```python
from build123d import *

# Parameters (mm, degrees)
BOSS_EXTRUDE1_DEPTH       = 28
CHAMFER1_SIZE             = 2
M8X1_0_TAPPED_HOLE1_D     = 7
M8X1_0_TAPPED_HOLE1_DEPTH = 13
M8X1_0_TAPPED_HOLE1_TIP   = 2.103012167
HOLE2_D                   = 9
SKETCH15_R                = 32.5
CUT_EXTRUDE3_DEPTH        = 2.5
CUT_EXTRUDE4_START        = -2.5
SKETCH16_R                = 32.5
CUT_EXTRUDE4_DEPTH        = 2.5
HOLE3_D                   = 4


with BuildPart() as part:
    # Sketch1 → Boss-Extrude1 (new body)
    with BuildSketch(Plane.XY):
        with BuildLine():
            Line((-50, 24), (-33, 24))
            Line((-33, 24), (-33, 47))
            Line((-33, 47), (33, 47))
            Line((33, 47), (33, 24))
            Line((33, 24), (50, 24))
            Line((50, 24), (50, 0))
            Line((50, 0), (30, 0))
            ThreePointArc((30, 0), (0, 30), (-30, 0))
            Line((-30, 0), (-50, 0))
            Line((-50, 0), (-50, 24))
        make_face()
    extrude(amount=BOSS_EXTRUDE1_DEPTH)

    # Chamfer1
    chamfer1_edges = [part.edges().sort_by_distance(p)[0] for p in [
        (-50, 24, 14),
        (-33, 47, 14),
        (33, 47, 14),
        (50, 24, 14),
    ]]
    chamfer(chamfer1_edges, length=CHAMFER1_SIZE)

    # M8x1.0 Tapped Hole1
    with Locations(Plane(origin=(0, 47, 0), x_dir=(1, 0, 0), z_dir=(0, 1, 0))):
        with Locations((0, -14)):
            Hole(M8X1_0_TAPPED_HOLE1_D / 2, depth=M8X1_0_TAPPED_HOLE1_DEPTH)
            with Locations((0, 0, -(M8X1_0_TAPPED_HOLE1_DEPTH + M8X1_0_TAPPED_HOLE1_TIP / 2))):  # 118° drill point
                Cone(0, M8X1_0_TAPPED_HOLE1_D / 2, M8X1_0_TAPPED_HOLE1_TIP, mode=Mode.SUBTRACT)

    # Hole2 (through all)
    with Locations(Plane(origin=(0, 24, 0), x_dir=(1, 0, 0), z_dir=(0, 1, 0))):
        with Locations((-41, -14), (41, -14)):
            Hole(HOLE2_D / 2)

    # Sketch15 → Cut-Extrude3 (cut)
    with BuildSketch(Plane(origin=(0, 0, 0), x_dir=(-1, 0, 0), z_dir=(0, 0, -1))):
        Circle(SKETCH15_R)
    extrude(amount=-CUT_EXTRUDE3_DEPTH, mode=Mode.SUBTRACT)

    # Sketch16 → Cut-Extrude4 (cut)
    with BuildSketch(Plane.XY.offset(28).offset(CUT_EXTRUDE4_START)):
        Circle(SKETCH16_R)
    extrude(amount=CUT_EXTRUDE4_DEPTH, mode=Mode.SUBTRACT)

    # Hole3 (through all)
    with Locations(Plane(origin=(0, 47, 0), x_dir=(1, 0, 0), z_dir=(0, 1, 0))):
        with Locations((0, -14)):
            Hole(HOLE3_D / 2)


solid = part.part
```
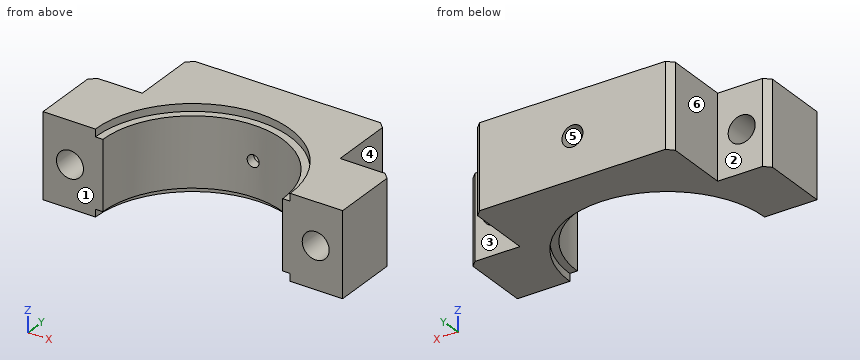
CAD build for the part. Positions are in the model's coordinates, mm. Face numbers are marked on the shaded views. A direction names the side the tool comes from. Coordinates: 2 decimals unless noted, no trailing zeros. Order: outer loops, then holes, each group sorted by start corner. A loop starts at its lowest first (then second) coordinate and runs counter-clockwise, first axis right, second up. Notation, with made-up numbers: (35, 55) - (72, 55) arc R21 cw to (72, 76) - close; hole circle Ø10 at (-11, 51.5). An arc over 180 degrees is marked (long way). Use a Markdown table: item, result. Add a question column.
(1) Pull direction X, two halves, no side cores. Call the marked faces 4, 5 and 6: +X half, -X half, draft (parallel to the pull), parting line (faces both ways), or undercut.
(2) Saw through at A-A (x = -41). Give the cut face in (y, z).
(3) Saw through at C-C (z = 14). Count the separate pieces of the cut face and the enclosed holes in it, then the cut area to 3 significant figures.
(4) Drill centre lines: line 1 along Z through (x, y) = (-41, 12); line 2 along X through (y, z) = (39, 17.75); line 3 along Z through (x, y) = (0, 32). Where is each one in solid material? Low to high. Write a range as [from, to].
(5) Flat gauge pins, fed straight in: pin 1 (10 mm diameter, centred on x = -15, y = 23, fed in from +Z); pin 2 (3 mm diameter, centred on x = -9.5, y = 26, fed in from -Z); pin 3 (10 mm diameter, centred on y = 36, z = 14, fed in from -X); pin 4 (5.5 mm diameter, centred on x = 0, z = 14, fed in from +Y). Where does each tip first touch, or does it go through?
(6) Which spindle directions (+Z, -Z, +X, -X, +Y, -Y) get a long thin tool onto all of the face, cutting with end or side? Do the marked faces 1, 2 and 3. Say none if no direction does.
(7) Saw through at B-B (y = 16.5). Give the cut face in (x, z), then the cut area to 3 significant figures.
(8) Saw through at D-D (y = 41). Give the cut face in (x, z).
Solved:
| question | item | result |
|---|---|---|
| 1 | face 4 | +X half |
| 1 | face 5 | undercut |
| 1 | face 6 | -X half |
| 2 | outline | (0, 0) - (24, 0) - (24, 9.5) - (0, 9.5) - close; (0, 18.5) - (24, 18.5) - (24, 28) - (0, 28) - close |
| 3 | separate pieces | 4 |
| 3 | enclosed holes | 0 |
| 3 | area | 1,960 mm² |
| 4 | line 1 | z = [0, 9.5], [18.5, 28] |
| 4 | line 2 | x = [-33, 33] |
| 4 | line 3 | z = [2.5, 12], [16, 25.5] |
| 5 | pin 1 | stops at z = 25.5 |
| 5 | pin 2 | passes through |
| 5 | pin 3 | stops at x = -33 |
| 5 | pin 4 | stops at y = 33.55 |
| 6 | face 1 | +Z, -Z, +X, -X, -Y |
| 6 | face 2 | +Z, -Z, -X, +Y |
| 6 | face 3 | +Z, -Z, +X, +Y |
| 7 | outline | (-50, 0) - (-28, 0) - (-28, 2.5) - (-25.05, 2.5) - (-25.05, 25.5) - (-28, 25.5) - (-28, 28) - (-50, 28) - close; (25.05, 2.5) - (28, 2.5) - (28, 0) - (50, 0) - (50, 28) - (28, 28) - (28, 25.5) - (25.05, 25.5) - close; hole circle Ø9 at (-41, 14); hole circle Ø9 at (41, 14) |
| 7 | area | 1,240 mm² |
| 8 | outline | (-33, 0) - (33, 0) - (33, 28) - (-33, 28) - close; hole circle Ø7 at (0, 14) |
